Verification items for the finished model (mm, model axes). A direction names the side the tool comes from. Round coordinates to 2 decimals unless told otherwise and drop trailing zeros. Order: outer loops, then holes, each group sorted by start corner. A loop starts at its lowest first (then second) coordinate and runs counter-clockwise, first axis right, second up. Notation, with made-up numbers: (22.5, -32.75) -> (45.5, -32.75) arc R12 cw to (45.5, -28.75) -> close; hole circle Ø11 at (56.25, -29.5). An arc over 180 degrees is marked (long way). Write item = value, one per line. Start each with the question number.
from build123d import *

# Parameters (mm, degrees)
SKETCH_1_W             = 70
SKETCH_1_H             = 101
EXTRUDE_1_DEPTH        = 12
SKETCH_2_R             = 15
CUT_EXTRUDE_1_DEPTH    = 7
SKETCH_3_R             = 12
CUT_EXTRUDE_2_DEPTH    = 124.085336251
CHAMFER_2_SIZE         = 0.5
HOLE_WIZARD_M6_1_D     = 5
HOLE_WIZARD_M6_1_DEPTH = 17
HOLE_WIZARD_M6_1_TIP   = 1.502151548
SKETCH_10_R            = 2.75
CUT_EXTRUDE_3_DEPTH    = 124.470644284


with BuildPart() as part:
    # 草图1 → 凸台-拉伸1 (new body)
    with BuildSketch(Plane.XY):
        with Locations((35, -50.5)):
            Rectangle(SKETCH_1_W, SKETCH_1_H)
    extrude(amount=EXTRUDE_1_DEPTH)

    # 草图2 → 切除-拉伸1 (cut)
    with BuildSketch(Plane.XY.offset(12)):
        with Locations((35, -51)):
            Circle(SKETCH_2_R)
    extrude(amount=-CUT_EXTRUDE_1_DEPTH, mode=Mode.SUBTRACT)

    # 草图3 → 切除-拉伸2 (cut, through all)
    with BuildSketch(Plane.XY.offset(5)):
        with Locations((35, -51)):
            Circle(SKETCH_3_R)
    extrude(amount=-CUT_EXTRUDE_2_DEPTH, mode=Mode.SUBTRACT)

    # 倒角2
    chamfer_2_edges = [part.edges().sort_by_distance(p)[0] for p in [
        (20, -51, 12),
    ]]
    chamfer(chamfer_2_edges, length=CHAMFER_2_SIZE)

    # M6 螺纹孔1
    with Locations(Plane(origin=(0, 0, 0), x_dir=(1, 0, 0), z_dir=(0, 1, 0))):
        with Locations((62.5, -6), (7.5, -6)):
            Hole(HOLE_WIZARD_M6_1_D / 2, depth=HOLE_WIZARD_M6_1_DEPTH)
            with Locations((0, 0, -(HOLE_WIZARD_M6_1_DEPTH + HOLE_WIZARD_M6_1_TIP / 2))):  # 118° drill point
                Cone(0, HOLE_WIZARD_M6_1_D / 2, HOLE_WIZARD_M6_1_TIP, mode=Mode.SUBTRACT)

    # 草图10 → 切除-拉伸3 (cut, through all)
    with BuildSketch(Plane(origin=(0, 0, 0), x_dir=(-1, 0, 0), z_dir=(0, 0, -1))):
        with Locations((-60, -96)):
            Circle(SKETCH_10_R)
        with Locations((-10, -96)):
            Circle(SKETCH_10_R)
    extrude(amount=-CUT_EXTRUDE_3_DEPTH, mode=Mode.SUBTRACT)


solid = part.part
(1) Depth check by flat-ended pin: pin 1 (24 mm diameter, centred on x = 36, y = -48.5, fed in from +Z). Enter the tip coordinate at first touch or a pass-through.
(2) Cross-section at B-B (x = 35). Enter the section's corners in (y, z), and give its area (3 significant figures).
(3) Draft check along X on faces 1 (the flat face through (19, -50, 12)), 2 (the flat face through (0, -51, 6)), 3 (the cylindrical face through (46.085, -55.596, 2.535)), 4 (the flat face through (70, -51, 6)). Enter one of: +X half, -X half, draft (parallel to the pull), parting line (faces both ways), or undercut.
(4) Cross-section at C-C (z = 7.5). Give the number of separate pieces and of enclosed holes in the cut face, and give its area (3 significant figures).
(5) Cross-section at A-A (z = 1.25). Enter the section's corners in (x, y).
(6) Scan lines: line 1 along Z through (x, y) = (62.5, -4.5); line 2 along Y through (x, z) = (35, 9); line 3 along Z through (x, y) = (35, -37.5). Record each from-to range of solid material in increasing order. Write a range as from..to.
(7) Set-up check for faces 5 (the cylindrical face through (9, -9, 4)), 6 (the flat face through (28, -41, 5)), 7 (the flat face through (35, 0, 6)): record each of +Z, -Z, +X, -X, +Y, -Y from which the full face is reachable in a straight line by a thin tool's end or side.
Outcome:
q1.pin_1 = 5
q2.outline = (-101, 0) -> (-63, 0) -> (-63, 5) -> (-66, 5) -> (-66, 11.5) -> (-66.5, 12) -> (-101, 12) -> close; (-39, 0) -> (0, 0) -> (0, 12) -> (-35.5, 12) -> (-36, 11.5) -> (-36, 5) -> (-39, 5) -> close
q2.area = 882 mm^2
q3.face_1 = draft
q3.face_2 = -X half
q3.face_3 = undercut
q3.face_4 = +X half
q4.separate_pieces = 1
q4.enclosed_holes = 3
q4.area = 6,180 mm^2
q5.outline = (0, -101) -> (70, -101) -> (70, 0) -> (0, 0) -> close; hole circle Ø5.5 at (10, -96); hole circle Ø24 at (35, -51); hole circle Ø5.5 at (60, -96)
q6.line_1 = 0..3.5, 8.5..12
q6.line_2 = -101..-66, -36..0
q6.line_3 = 0..5
q7.face_5 = +Y
q7.face_6 = +Z
q7.face_7 = +Z, -Z, +X, -X, +Y
